```python
from build123d import *

# Parameters (mm, degrees)
BOSS_EXTRUDE1_DEPTH = 11.5
SKETCH4_R           = 12.5
BOSS_EXTRUDE2_DEPTH = 18
SKETCH5_R           = 20
BOSS_EXTRUDE3_DEPTH = 5
SKETCH6_R           = 14
BOSS_EXTRUDE4_DEPTH = 2
SKETCH7_R           = 17.5
BOSS_EXTRUDE5_DEPTH = 8
SKETCH8_R           = 11
CUT_EXTRUDE1_DEPTH  = 28
SKETCH9_R           = 10
CUT_EXTRUDE2_DEPTH  = 71


with BuildPart() as part:
    # Sketch1 → Boss-Extrude1 (new, symmetric)
    with BuildSketch(Plane.XY):
        Polygon((0, 28.867513459), (-25, 14.43375673), (-25, -14.43375673), (0, -28.867513459), (25, -14.43375673), (25, 14.43375673), align=None)
    extrude(amount=BOSS_EXTRUDE1_DEPTH, both=True)

    # Sketch3 → Cut-Revolve1 (revolve, cut)
    with BuildSketch(Plane(origin=(0, 0, 0), x_dir=(0, 0, -1), z_dir=(1, 0, 0)), mode=Mode.PRIVATE) as cut_revolve1_sk:
        Polygon((11.5, 12.5), (3.5, 28.867513459), (11.5, 28.867513459), align=None)
    revolve(cut_revolve1_sk.sketch.rotate(Axis((0, 0, 1000), (0, 0, -1)), 90), axis=Axis((0, 0, 1000), (0, 0, -1)), mode=Mode.SUBTRACT)

    # Sketch4 → Boss-Extrude2 (add)
    with BuildSketch(Plane(origin=(0, 0, -11.5), x_dir=(-1, 0, 0), z_dir=(0, 0, -1))):
        Circle(SKETCH4_R)
    extrude(amount=BOSS_EXTRUDE2_DEPTH)

    # Sketch5 → Boss-Extrude3 (add)
    with BuildSketch(Plane.XY.offset(11.5)):
        Circle(SKETCH5_R)
    extrude(amount=BOSS_EXTRUDE3_DEPTH)

    # Sketch6 → Boss-Extrude4 (add)
    with BuildSketch(Plane.XY.offset(16.5)):
        Circle(SKETCH6_R)
    extrude(amount=BOSS_EXTRUDE4_DEPTH)

    # Sketch7 → Boss-Extrude5 (add)
    with BuildSketch(Plane.XY.offset(18.5)):
        Circle(SKETCH7_R)
    extrude(amount=BOSS_EXTRUDE5_DEPTH)

    # Sketch8 → Cut-Extrude1 (cut)
    with BuildSketch(Plane.XY.offset(26.5)):
        Circle(SKETCH8_R)
    extrude(amount=-CUT_EXTRUDE1_DEPTH, mode=Mode.SUBTRACT)

    # Sketch9 → Cut-Extrude2 (cut)
    with BuildSketch(Plane(origin=(0, 0, -29.5), x_dir=(-1, 0, 0), z_dir=(0, 0, -1))):
        Circle(SKETCH9_R)
    extrude(amount=-CUT_EXTRUDE2_DEPTH, mode=Mode.SUBTRACT)


solid = part.part
```
Here's how the part is built. I have some questions about the finished solid (model axes, mm). A direction names the side the tool comes from. Coordinates: 2 decimals unless noted, no trailing zeros. Order: outer loops, then holes, each group sorted by start corner. A loop starts at its lowest first (then second) coordinate and runs counter-clockwise, first axis right, second up. Notation, with made-up numbers: M 64.5,-3.75 L 79.5,-3.75 A21 cw 79.5,16.25 Z; hole C -8,43.25 d3. An arc over 180 degrees is marked long. Answer as a JSON object with one key per item and string values. Group by question number.
(1) Which directions (+Z, -Z, +X, -X, +Y, -Y) give clear straight access to the entire face, cutting with the end or side of a thin tool? Please do faces 1 (the face through (-8, 12, 18.5)), 2 (the face through (12.675, 21.55, 3.173)), 3 (the face through (-25, 0, 3)), 4 (the face through (-11.923, 3.755, -20.374)), 5 (the face through (-13.887, -10.648, 22.444)).
(2) I need wall thicknesses on probe 1 along Y at (x, z) = (0, -23.5); probe 2 along Y at (x, z) = (0, 20.25); probe 3 along Z at (x, y) = (10.5, 10). Which ranges of each line are inside material? Lowest first, please.
(3) If we mould it in two halves opening along X, with no side actions, what happens to faces 6 (the face through (12.9, -4.06, -11)), 7 (the face through (2.17, -9.76, -15.7)), 8 (the face through (-14, -4, 16.5)), 9 (the face through (-2.38, -10.74, 12.7))? For each: released by +X, released by -X, zero draft, split by the parting line, or undercut.
(4) Suppose I cut it at A-A, the plane z = 1. Please give me the cut outline in (x, y), then the cut area to 3 significant figures.
(5) For pin 1 (18 mm diameter, centred on x = 0, y = 0, fed in from -Z); pin 2 (10 mm diameter, centred on x = -14.5, z = 5.5, fed in from -Y); pin 3 (1 mm diameter, centred on x = -18.5, y = -16, fed in from +Z); pin 4 (4 mm diameter, centred on y = -16.5, z = 20.5, fed in from +X), each with a flat end and sliding along its axis, tell me the tip position at first contact or that it passes through.
(6) Suppose I cut it at B-B, the plane y = 0. Please give me the cut outline in (x, z).
Values found:
{
 "1": {"face 1": "none", "face 2": "+Z, -Z, +X, +Y", "face 3": "+Z, -Z, -X, +Y, -Y", "face 4": "-Z", "face 5": "+Z"},
 "2": {"probe 1": "y = -12.5 to -10, 10 to 12.5", "probe 2": "y = -17.5 to -11, 11 to 17.5", "probe 3": "z = -10.52 to 16.5, 18.5 to 26.5"},
 "3": {"face 6": "split by the parting line", "face 7": "undercut", "face 8": "zero draft", "face 9": "undercut"},
 "4": {"outline": "M -25,-14.43 L 0,-28.87 L 25,-14.43 L 25,14.43 L 0,28.87 L -25,14.43 Z; hole C 0,0 d22", "area": "1,780 mm^2"},
 "5": {"pin 1": "passes through", "pin 2": "stops at y = -23.38", "pin 3": "stops at z = 11.5", "pin 4": "stops at x = 9.8"},
 "6": {"outline": "M -25,-5.39 L -12.5,-11.5 L -12.5,-29.5 L -10,-29.5 L -10,-1.5 L -11,-1.5 L -11,26.5 L -17.5,26.5 L -17.5,18.5 L -14,18.5 L -14,16.5 L -20,16.5 L -20,11.5 L -25,11.5 Z; M 10,-29.5 L 12.5,-29.5 L 12.5,-11.5 L 25,-5.39 L 25,11.5 L 20,11.5 L 20,16.5 L 14,16.5 L 14,18.5 L 17.5,18.5 L 17.5,26.5 L 11,26.5 L 11,-1.5 L 10,-1.5 Z"}
}
